Verification items for the finished model (mm, model axes). Face numbers are marked on the shaded views. A direction names the side the tool comes from. Round coordinates to 2 decimals unless told otherwise and drop trailing zeros. Write each loop counter-clockwise with the first axis right and the second up, starting at its lowest first coordinate (ties: lowest second). Pieces come first, ordered by that corner, then holes. Notation, with made-up numbers: M 76,80 L 95,80 A20 cw 95,85 Z; hole C 69.5,75.25 d9. An arc over 180 degrees is marked long. One line per item, written item: value. Start each with the question number.
Item 1: Draft check along Y on the marked faces 1, 2, 3 and 4. Enter one of: +Y half, -Y half, draft (parallel to the pull), parting line (faces both ways), or undercut.
Item 2: Tool access check on the marked faces 5, 6 and 7. Record the directions out of +Z, -Z, +X, -X, +Y, -Y that give a thin tool (end or side, any length) a straight path to the whole face; none if there is none.
Item 3: Section check C-C, the plane z = -12. State how many separate pieces and enclosed holes the cut face has, then the cut area to 3 significant figures.
Item 4: Section check A-A, the plane x = -18. Record the cut outline in (y, z), then the cut area to 3 significant figures.
Item 5: Thickness scan on probe 1 along X at (y, z) = (2.5, -18); probe 2 along Z at (x, y) = (-18, 3.5); probe 3 along X at (y, z) = (4.25, 19). Record the ranges inside material, lowest first. Write a range as from..to.
Item 6: Section check B-B, the plane z = -18. Record the cut outline in (x, y), then the cut area to 3 significant figures.
Item 7: Gauge pin test, flat ends, axial feed: pin 1 (2 mm diameter, centred on x = -5, z = 10, fed in from +Y); pin 2 (16.5 mm diameter, centred on x = 12, z = -2.5, fed in from +Y); pin 3 (1.5 mm diameter, centred on y = 1, z = -14.5, fed in from +X); pin 4 (2.5 mm diameter, centred on x = 18, z = 18, fed in from +Y). Record the tip position at first contact, or that the pin passes through.
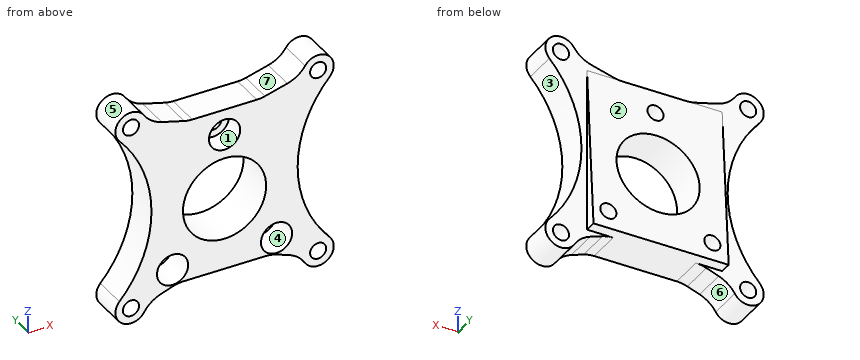
from build123d import *

# Parameters (mm, degrees)
SKETCH_1_R           = 1.55
EXTRUDE_1_DEPTH      = 6.5
EXTRUDE_2_DEPTH      = 13
EXTRUDE_2_DEPTH_BACK = 13
FILLET_1_R           = 6
SKETCH_5_R           = 1.55
SKETCH_5_R_2         = 8
CUT_EXTRUDE_3_DEPTH  = 32.013570632
SKETCH_6_R           = 3
CUT_EXTRUDE_10_DEPTH = 6


with BuildPart() as part:
    # 草图1 → 凸台-拉伸1 (new body)
    with BuildSketch(Plane(origin=(0, 0, 0), x_dir=(1, 0, 0), z_dir=(0, 1, 0))):
        with BuildLine():
            Line((-15, 18), (-9, 15.85))
            Line((-9, 15.85), (9, 15.85))
            Line((9, 15.85), (15, 18))
            ThreePointArc((15, 18), (19.079157226, 20.799181966), (20.223613121, 15.986161702))
            ThreePointArc((20.223613121, 15.986161702), (14.060533289, 0), (20.223613121, -15.986161702))
            ThreePointArc((20.223613121, -15.986161702), (19.079157226, -20.799181966), (15, -18))
            Line((15, -18), (7, -15.85))
            Line((7, -15.85), (-7, -15.85))
            Line((-7, -15.85), (-15, -18))
            ThreePointArc((-15, -18), (-19.079157226, -20.799181966), (-20.223613121, -15.986161702))
            ThreePointArc((-20.223613121, -15.986161702), (-14.060533289, 0), (-20.223613121, 15.986161702))
            ThreePointArc((-20.223613121, 15.986161702), (-19.079157226, 20.799181966), (-15, 18))
        make_face()
        with Locations(Location((18, 18, 0), (0, 0, 90))):
            Circle(SKETCH_1_R, mode=Mode.SUBTRACT)
        with Locations(Location((18, -18, 0), (0, 0, 90))):
            Circle(SKETCH_1_R, mode=Mode.SUBTRACT)
        with Locations(Location((-18, -18, 0), (0, 0, 90))):
            Circle(SKETCH_1_R, mode=Mode.SUBTRACT)
        with Locations(Location((-18, 18, 0), (0, 0, 90))):
            Circle(SKETCH_1_R, mode=Mode.SUBTRACT)
    extrude(amount=EXTRUDE_1_DEPTH)

    # 草图3 → 凸台-拉伸2 (add, two sides: drawn at the far end of the back side and taken through both)
    with BuildSketch(Plane(origin=(0, 0, 0), x_dir=(0, 0, -1), z_dir=(1, 0, 0)).offset(-EXTRUDE_2_DEPTH_BACK)):
        Polygon((-15.85, 6.5), (15.85, 6.5), (15.85, 8.716679939), align=None)
    extrude(amount=EXTRUDE_2_DEPTH + EXTRUDE_2_DEPTH_BACK)

    # 圆角1
    fillet_1_edges = [part.edges().sort_by_distance(p)[0] for p in [
        (15, 3.25, 18),
        (7, 3.25, 15.85),
        (-7, 3.25, 15.85),
        (-15, 3.25, 18),
        (-15, 3.25, -18),
        (-9, 3.25, -15.85),
        (9, 3.25, -15.85),
        (15, 3.25, -18),
    ]]
    fillet(fillet_1_edges, radius=FILLET_1_R)

    # 草图5 → 切除-拉伸3 (cut, through all)
    with BuildSketch(Plane(origin=(0, 7.571318049, 0.529438133), x_dir=(1, 0, 0), z_dir=(0, 0.9975640502598243, 0.06975647374412569))):
        with Locations(Location((10, 12.85, 0), (0, 0, 270))):
            Circle(SKETCH_5_R)
        with Locations(Location((0, -10.85, 0), (0, 0, 270))):
            Circle(SKETCH_5_R)
        with Locations(Location((-10, 12.85, 0), (0, 0, 270))):
            Circle(SKETCH_5_R)
        with Locations(Location((0, 1.85, 0), (0, 0, 270))):
            Circle(SKETCH_5_R_2)
    extrude(amount=-CUT_EXTRUDE_3_DEPTH, mode=Mode.SUBTRACT)

    # 草图6 → 切除-拉伸10 (cut)
    with BuildSketch(Plane(origin=(0, 1.528635135, -42.076453462), x_dir=(-1, 0, 0), z_dir=(0, 0.9975640502598243, 0.06975647374412568))):
        with Locations(Location((0, 52.930589533, 0), (0, 0, 270))):
            Circle(SKETCH_6_R)
        with Locations(Location((10, 29.230589533, 0), (0, 0, 270))):
            Circle(SKETCH_6_R)
        with Locations(Location((-10, 29.230589533, 0), (0, 0, 270))):
            Circle(SKETCH_6_R)
    extrude(amount=CUT_EXTRUDE_10_DEPTH, mode=Mode.SUBTRACT)


solid = part.part
Response values:
1. face 1: undercut
1. face 2: +Y half
1. face 3: draft
1. face 4: undercut
2. face 5: +Y, -Y
2. face 6: -Z, +Y, -Y
2. face 7: +Z, +Y, -Y
3. separate pieces: 3
3. enclosed holes: 0
3. area: 194 mm2
4. outline: M 0,-21 L 6.5,-21 L 6.5,-19.55 L 0,-19.55 Z; M 0,-16.45 L 6.5,-16.45 L 6.5,-13.12 L 0,-13.12 Z; M 0,13.12 L 6.5,13.12 L 6.5,16.45 L 0,16.45 Z; M 0,19.55 L 6.5,19.55 L 6.5,21 L 0,21 Z
4. area: 62.2 mm2
5. probe 1: x = -21..-19.55, -16.45..-14.06, 14.06..16.45, 19.55..21
5. probe 2: z = -21..-19.55, -16.45..-13.12, 13.12..16.45, 19.55..21
5. probe 3: x = -20.83..-19.18, -16.82..-14.99, 14.99..16.82, 19.18..20.83
6. outline: M -21,0 L -19.55,0 L -19.55,6.5 L -21,6.5 Z; M -16.45,0 L -14.06,0 L -14.06,6.5 L -16.45,6.5 Z; M 14.06,0 L 16.45,0 L 16.45,6.5 L 14.06,6.5 Z; M 19.55,0 L 21,0 L 21,6.5 L 19.55,6.5 Z
6. area: 50.0 mm2
7. pin 1: stops at y = 6.98
7. pin 2: stops at y = 8.36
7. pin 3: stops at x = 19.58
7. pin 4: passes through
